Input: part model. Units: mm. Frame: model coordinates. Face numbers are marked on the shaded views. A direction names the side the tool comes from. Give positions to 0.01 mm unless a question says otherwise; leave off trailing zeros. Order: outer loops, then holes, each group sorted by start corner. A loop starts at its lowest first (then second) coordinate and runs counter-clockwise, first axis right, second up. Notation, with made-up numbers: M 38,74 L 57,74 A22 ccw 57,105 Z; hole C 68,83.25 d7. An arc over 180 degrees is marked long. Use a Markdown table: item, result.
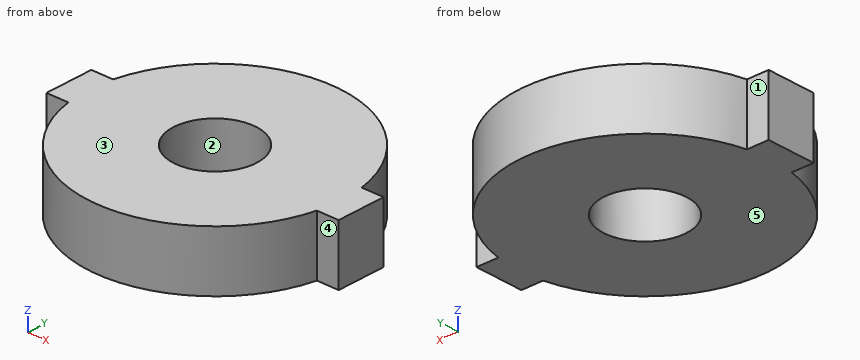
from build123d import *

# Parameters (mm, degrees)
SKETCH1_R           = 4.25
BOSS_EXTRUDE1_DEPTH = 6


with BuildPart() as part:
    # Sketch1 → Boss-Extrude1 (new body)
    with BuildSketch(Plane.XY.offset(6)):
        with BuildLine():
            Line((-12.757350822, 2.5), (-15, 2.5))
            Line((-15, 2.5), (-15, -2.5))
            Line((-15, -2.5), (-12.757350822, -2.5))
            ThreePointArc((-12.757350822, -2.5), (0, -13), (12.757350822, -2.5))
            Line((12.757350822, -2.5), (15, -2.5))
            Line((15, -2.5), (15, 2.5))
            Line((15, 2.5), (12.757350822, 2.5))
            ThreePointArc((12.757350822, 2.5), (0, 13), (-12.757350822, 2.5))
        make_face()
        with Locations(Location((0, 0, 0), (0, 0, 180))):
            Circle(SKETCH1_R, mode=Mode.SUBTRACT)
    extrude(amount=-BOSS_EXTRUDE1_DEPTH)


solid = part.part
1) Material intervals for line 1 (X direction, y = 0.25, z = 1.2); line 2 (Y direction, x = 0.5, z = 4.95); line 3 (X direction, y = 4.75, z = 0.55), sorted ascending. Write a range as from..to.
Response values:
| item | result |
|---|---|
| line 1 | x = -15..-4.24, 4.24..15 |
| line 2 | y = -12.99..-4.22, 4.22..12.99 |
| line 3 | x = -12.1..12.1 |
2) Cut plane C-C on y = 0. Return loops of the section in (x, z).
Response values:
| item | result |
|---|---|
| outline | M -15,0 L -4.25,0 L -4.25,6 L -15,6 Z; M 4.25,0 L 15,0 L 15,6 L 4.25,6 Z |
3) First-contact query: pin 1 Ø0.7 at (x, z) = (13.5, 2) entering from +Y; pin 2 Ø1.8 at (x, z) = (14, 4) entering from -Y; pin 3 Ø1 at (y, z) = (-6, 4.5) entering from +X. Flat tips, straight axial feed; report the tip coordinate or a pass-through.
Response values:
| item | result |
|---|---|
| pin 1 | stops at y = 2.5 |
| pin 2 | stops at y = -2.5 |
| pin 3 | stops at x = 11.78 |
4) Mould query, pull axis Y, two halves, no side actions, for the marked faces 1, 2 and 3. Classes: released by +Y, released by -Y, zero draft, split by the parting line, or undercut.
Response values:
| item | result |
|---|---|
| face 1 | released by +Y |
| face 2 | undercut |
| face 3 | zero draft |
5) Cut plane D-D on y = 5. Return loops of the section in (x, z), and give its area (3 significant figures).
Response values:
| item | result |
|---|---|
| outline | M -12,0 L 12,0 L 12,6 L -12,6 Z |
| area | 144 mm² |
6) Cut plane A-A on z = 3. Return loops of the section in (x, y).
Response values:
| item | result |
|---|---|
| outline | M -15,-2.5 L -12.76,-2.5 A13 ccw 12.76,-2.5 L 15,-2.5 L 15,2.5 L 12.76,2.5 A13 ccw -12.76,2.5 L -15,2.5 Z; hole C 0,0 d8.5 |
7) Cut plane B-B on x = 0. Return loops of the section in (y, z).
Response values:
| item | result |
|---|---|
| outline | M -13,0 L -4.25,0 L -4.25,6 L -13,6 Z; M 4.25,0 L 13,0 L 13,6 L 4.25,6 Z |
8) Reachability of the marked faces 4 and 5 from +Z, -Z, +X, -X, +Y, -Y: full face, straight path, thin tool, end or side. Return the list, or none.
Response values:
| item | result |
|---|---|
| face 4 | +Z, -Z, +X, -Y |
| face 5 | -Z, +X, -X, +Y, -Y |
